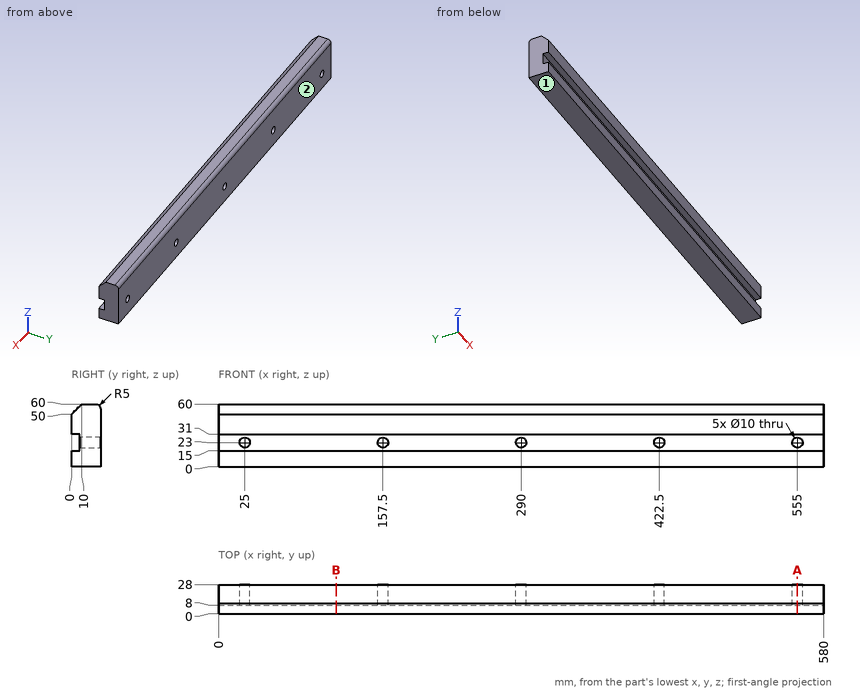
Input: dimensioned drawing with shaded views. Units: mm. Origin: part minimum x, y, z. Give positions to 0.01 mm unless a question says otherwise; leave off trailing zeros. Order: outer loops, then holes, each group sorted by start corner. A loop starts at its lowest first (then second) coordinate and runs counter-clockwise, first axis right, second up. Notation, with made-up numbers: (-30.5, -24.5) -> (10.5, -24.5) arc R22 cw to (10.5, -9.5) -> close; hole circle Ø4 at (85, 48). An arc over 180 degrees is marked (long way). Answer as a JSON object with one key per item and string values.
Q1. First-contact query: pin 1 (4 mm diameter, centred on x = 265.5, y = 6, fed in from +Z); pin 2 (5 mm diameter, centred on x = 435, z = 20.5, fed in from -Y). Flat tips, straight axial feed; report the tip coordinate or a pass-through.
Entries:
{"pin 1": "stops at z = 58", "pin 2": "stops at y = 8"}
Q2. Material intervals for probe 1 along X at (y, z) = (19.5, 23); probe 2 along X at (y, z) = (23.25, 22); probe 3 along Z at (x, y) = (290, 16.75), sorted ascending.
Entries:
{"probe 1": "x = 0 to 20, 30 to 152.5, 162.5 to 285, 295 to 417.5, 427.5 to 550, 560 to 580", "probe 2": "x = 0 to 20.1, 29.9 to 152.6, 162.4 to 285.1, 294.9 to 417.6, 427.4 to 550.1, 559.9 to 580", "probe 3": "z = 0 to 18, 28 to 60"}
Q3. Section B-B (x = 112.5). Output: boundary loops of the cut face in (y, z).
Entries:
{"outline": "(0, 0) -> (28, 0) -> (28, 55) arc R5 ccw to (23, 60) -> (10, 60) -> (0, 50) -> (0, 31) -> (8, 31) -> (8, 15) -> (0, 15) -> close"}
Q4. Section A-A (x = 555). Output: boundary loops of the cut face in (y, z), plus the area to 3 significant figures.
Entries:
{"outline": "(0, 0) -> (28, 0) -> (28, 18) -> (8, 18) -> (8, 15) -> (0, 15) -> close; (0, 31) -> (8, 31) -> (8, 28) -> (28, 28) -> (28, 55) arc R5 ccw to (23, 60) -> (10, 60) -> (0, 50) -> close", "area": "1,300 mm^2"}
Q5. Draft query along Y for the marked faces 1 and 2. Return one class per face: released by +Y, released by -Y, zero draft, split by the parting line, or undercut.
Entries:
{"face 1": "zero draft", "face 2": "released by +Y"}
